Read the model definition and answer for the solid it produces. Units are mm, in the model's axes. A direction names the side the tool comes from. Coordinates: 2 decimals unless noted, no trailing zeros. Loops run counter-clockwise (first coordinate to the right, second up) from the corner with the lowest first, then second, coordinate; pieces in that order, holes last. Notation, with made-up numbers: M 45.5,44.5 L 97.5,44.5 A20 cw 97.5,68.5 Z; hole C -37,41.25 d5. An arc over 180 degrees is marked long. One line per item, written item: value. Start each with the question number.
1. Consider probe 1 along Y at (x, z) = (19.5, -3); probe 2 along X at (y, z) = (0.5, 6.5). Determine where each line is inside the solid, lowest interval first.
2. The part is cut by section B-B (x = 29). Write down the section's boundary in (y, z), then the cut area to 3 significant figures.
3. For faces 4 (the face through (3, 0, -9)), 5 (the face through (7.5, -6, -2.4)), determine the directions among +Z, -Z, +X, -X, +Y, -Y from which every point of the face is accessible in a straight line to the end or side of a thin tool.
4. Flat-ended cylindrical pins translate along their axes: pin 1 (4 mm diameter, centred on x = 31, y = -7.5, fed in from -Z); pin 2 (6 mm diameter, centred on x = 23, y = 7.5, fed in from +Z); pin 3 (12 mm diameter, centred on x = 32.5, y = -2, fed in from -Z). Find the tip coordinate at first contact, or state that the pin passes through.
5. The part is cut by section A-A (x = 2). Write down the section's boundary in (y, z).
6. Determine the mould class of faces 1 (the face through (9.695, 1.214, 5.465)), 2 (the face through (0.19, 4.65, 8.09)), 3 (the face through (3.4, -7.83, -4.44)) for opening direction X: +X half, -X half, draft (parallel to the pull), parting line (faces both ways), or undercut.
```python
from build123d import *

# Parameters (mm, degrees)
EXTRUDE_1_DEPTH     = 7.5
SKETCH_4_R          = 20.03
SKETCH_4_R_2        = 9
CUT_EXTRUDE_1_DEPTH = 0.9375
CUT_EXTRUDE_1_DRAFT = -60
CHAMFER_1_SIZE      = 0.666666667


with BuildPart() as part:
    # 草图3 → 凸台-拉伸1 (new body)
    with BuildSketch(Plane(origin=(0, 0, 0), x_dir=(0, 0, -1), z_dir=(1, 0, 0))):
        Polygon((9, 5.196152423), (0, 10.392304845), (-9, 5.196152423), (-9, -5.196152423), (0, -10.392304845), (9, -5.196152423), align=None)
    extrude(amount=EXTRUDE_1_DEPTH)


with BuildPart() as cut_extrude_1_tool:
    # 草图4 → 切除-拉伸1 (with draft: the straight prism first)
    with BuildSketch(Plane.ZY):
        Circle(SKETCH_4_R)
        Circle(SKETCH_4_R_2, mode=Mode.SUBTRACT)
    extrude(amount=-CUT_EXTRUDE_1_DEPTH)
    # 切除-拉伸1: the draft: its side faces are tilted about the plane it starts from
    cut_extrude_1_sides = [cut_extrude_1_tool.faces().sort_by_distance(p)[0] for p in [
        (0.46875, 0, -20.03),
        (0.46875, 0, -9),
    ]]
    draft(cut_extrude_1_sides, Plane.ZY, CUT_EXTRUDE_1_DRAFT)


with BuildPart() as part_1:
    add(part.part)

    # 切除-拉伸1: cut by cut_extrude_1_tool
    add(cut_extrude_1_tool.part, mode=Mode.SUBTRACT)

    # 草图6 → 旋转2 (revolve)
    with BuildSketch(Plane.XY, mode=Mode.PRIVATE) as revolve_2_sk:
        with BuildLine():
            Line((12.8, 6), (37.5, 6))
            Line((37.5, 6), (37.5, 0))
            Line((37.5, 0), (7.5, 0))
            Line((7.5, 0), (7.5, 6.2816875))
            ThreePointArc((7.5, 6.2816875), (7.788817563, 5.643272061), (8.458998289, 5.438705073))
            Line((8.458998289, 5.438705073), (12.8, 6))
        make_face()
    revolve(revolve_2_sk.sketch.rotate(Axis((7.5, 0, 0), (1, 0, 0)), 180), axis=Axis((7.5, 0, 0), (1, 0, 0)))

    # 倒角1
    chamfer_1_edges = [part_1.edges().sort_by_distance(p)[0] for p in [
        (37.5, 6, 0),
    ]]
    chamfer(chamfer_1_edges, length=CHAMFER_1_SIZE)

    # 草图8 → 切除-旋转2 (revolve, cut)
    with BuildSketch(Plane.XY, mode=Mode.PRIVATE) as cut_revolve_2_sk:
        Polygon((7.5, 8.215), (6.9, 8.815), (6.9, 20.03), (7.5, 20.03), align=None)
    revolve(cut_revolve_2_sk.sketch.rotate(Axis((0, 0, 0), (1, 0, 0)), 180), axis=Axis((0, 0, 0), (1, 0, 0)), mode=Mode.SUBTRACT)


solid = part_1.part
```
Answer block:
1. probe 1: y = -5.2 to 5.2
1. probe 2: x = 0 to 7.5
2. outline: C 0,0 d12
2. area: 113 mm2
3. face 4: -Z, +X, -X, +Y, -Y
3. face 5: +X
4. pin 1: stops at z = -2.4
4. pin 2: stops at z = 3.97
4. pin 3: stops at z = -6
5. outline: M -10.39,0 L -5.2,-9 L 5.2,-9 L 10.39,0 L 5.2,9 L -5.2,9 Z
6. face 1: undercut
6. face 2: -X half
6. face 3: draft
